```python
from build123d import *

# Parameters (mm, degrees)
SKETCH2_R           = 1.25
BOSS_EXTRUDE1_DEPTH = 1.5


with BuildPart() as part:
    # Sketch2 → Boss-Extrude1 (new body)
    with BuildSketch(Plane(origin=(0, 0, 0), x_dir=(1, 0, 0), z_dir=(0, 1, 0))):
        with BuildLine():
            Line((-10.401091034, -13.320036445), (-9.505079721, -12.172569963))
            ThreePointArc((-9.505079721, -12.172569963), (-5.62952549, -11.294814862), (-3.997208572, -14.91778548))
            Line((-3.997208572, -14.91778548), (-4.891679952, -18.255998117))
            ThreePointArc((-4.891679952, -18.255998117), (0, 18.9), (4.891679952, -18.255998117))
            Line((4.891679952, -18.255998117), (3.997208572, -14.91778548))
            ThreePointArc((3.997208572, -14.91778548), (5.62952549, -11.294814862), (9.505079721, -12.172569963))
            Line((9.505079721, -12.172569963), (10.401091034, -13.320036445))
            ThreePointArc((10.401091034, -13.320036445), (0, 15.3), (-10.401091034, -13.320036445))
        make_face()
        with Locations(Location((-7.030215667, -14.105093678, 0), (0, 0, 270))):
            Circle(SKETCH2_R, mode=Mode.SUBTRACT)
        with Locations(Location((7.030215667, -14.105093678, 0), (0, 0, 90))):
            Circle(SKETCH2_R, mode=Mode.SUBTRACT)
    extrude(amount=BOSS_EXTRUDE1_DEPTH)


solid = part.part
```
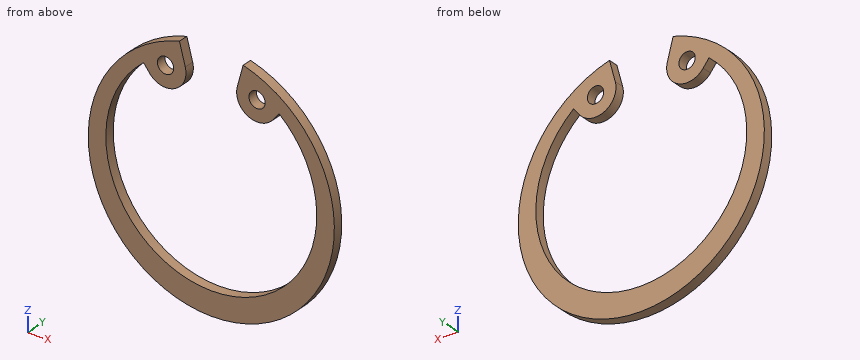
The model under review builds one solid part; all positions refer to its coordinate system, in mm. Round coordinates to 2 decimals unless told otherwise and drop trailing zeros. Order: outer loops, then holes, each group sorted by start corner. A loop starts at its lowest first (then second) coordinate and runs counter-clockwise, first axis right, second up. Notation, with made-up numbers: (43, 49.5) - (81, 49.5) arc R22 ccw to (81, 83.5) - close; hole circle Ø4 at (64, 50.25). An arc over 180 degrees is marked (long way). Answer in a Markdown table with one row per item.
(1) Clearance check with a flat-ended pin moving along its axis: P1, Ø1.5, axis at x = -7.03, z = 14.11, coming from the -Y side. State where the tip first meets the part, or that it passes through.
Result set:
| item | result |
|---|---|
| P1 | passes through |
(2) Take a section at A-A on z = -1.5. Write out the cut boundary in (x, y).
Result set:
| item | result |
|---|---|
| outline | (-18.84, 0) - (-16.02, 0) - (-16.02, 1.5) - (-18.84, 1.5) - close; (16.02, 0) - (18.84, 0) - (18.84, 1.5) - (16.02, 1.5) - close |
(3) Take a section at C-C on x = 6.5. Write out the cut boundary in (y, z), plus the area to 3 significant figures.
Result set:
| item | result |
|---|---|
| outline | (0, -17.75) - (1.5, -17.75) - (1.5, -13.94) - (0, -13.94) - close; (0, 11.01) - (1.5, 11.01) - (1.5, 12.97) - (0, 12.97) - close; (0, 15.24) - (1.5, 15.24) - (1.5, 17.75) - (0, 17.75) - close |
| area | 12.4 mm2 |
(4) Take a section at B-B on x = -14. Write out the cut boundary in (y, z).
Result set:
| item | result |
|---|---|
| outline | (0, -12.7) - (1.5, -12.7) - (1.5, -7.25) - (0, -7.25) - close; (0, 9.05) - (1.5, 9.05) - (1.5, 12.7) - (0, 12.7) - close |
(5) Take a section at D-D on y = 0.75. Write out the cut boundary in (x, z).
Result set:
| item | result |
|---|---|
| outline | (-10.4, 13.32) - (-9.51, 12.17) arc R3.14 ccw to (-4, 14.92) - (-4.89, 18.26) arc R18.9 ccw (long way) to (4.89, 18.26) - (4, 14.92) arc R3.14 ccw to (9.51, 12.17) - (10.4, 13.32) arc R16.2 cw (long way) to start; hole circle Ø2.5 at (-7.03, 14.11); hole circle Ø2.5 at (7.03, 14.11) |
(6) For line 1 (X direction, y = 0.3, z = 15); line 2 (X direction, y = 0.6, z = 13.5); line 3 (X direction, y = 1.3, z = -10), list the stretches that pass through material, from the lowest coordinate up. Write a range as from..to.
Result set:
| item | result |
|---|---|
| line 1 | x = -11.5..-7.9, -6.16..-4.02, 4.02..6.16, 7.9..11.5 |
| line 2 | x = -13.23..-8.12, -5.94..-3.95, 3.95..5.94, 8.12..13.23 |
| line 3 | x = -16.04..-11.98, 11.98..16.04 |
